from build123d import *

# Parameters (mm, degrees)
SKETCH1_R              = 1.6
BOSS_EXTRUDE1_DEPTH    = 4
CUT_EXTRUDE1_DEPTH     = 44.119746057
R1_CUTOUT_FILLET_R     = 1
R3_OUTER_EDGE_FILLET_R = 3


with BuildPart() as part:
    # Sketch1 → Boss-Extrude1 (new body)
    with BuildSketch(Plane(origin=(0, 0, 0), x_dir=(1, 0, 0), z_dir=(0, 1, 0))):
        Polygon((-40.5, -4.5), (-22.92820323, -4.5), (-16, -0.5), (16, -0.5), (22.92820323, -4.5), (40.5, -4.5), (40.5, 4), (26, 4), (5.5, 14.25), (-5.5, 14.25), (-26, 4), (-40.5, 4), align=None)
        with Locations(Location((-36, 0, 0), (0, 0, 270))):
            Circle(SKETCH1_R, mode=Mode.SUBTRACT)
        with Locations(Location((36, 0, 0), (0, 0, 270))):
            Circle(SKETCH1_R, mode=Mode.SUBTRACT)
        with Locations(Location((0, 10.25, 0), (0, 0, 270))):
            Circle(SKETCH1_R, mode=Mode.SUBTRACT)
    extrude(amount=BOSS_EXTRUDE1_DEPTH)

    # Sketch2 → Cut-Extrude1 (cut, through all)
    with BuildSketch(Plane(origin=(0, 4, 0), x_dir=(1, 0, 0), z_dir=(0, 1, 0))):
        Polygon((-7.655238394, 9.259261842), (-21.173762079, 2.5), (-3.75277675, 2.5), align=None)
        Polygon((-2.742413779, 6.75), (0, 2), (2.742413779, 6.75), align=None)
        Polygon((21.173762079, 2.5), (3.75277675, 2.5), (7.655238394, 9.259261842), align=None)
        Polygon((-31.5, 0), (-21.133974596, 0), (-25.464101615, -2.5), (-31.5, -2.5), align=None)
        Polygon((25.464101615, -2.5), (31.5, -2.5), (31.5, 0), (21.133974596, 0), align=None)
    extrude(amount=-CUT_EXTRUDE1_DEPTH, mode=Mode.SUBTRACT)

    # R1 cutout fillet
    r1_cutout_fillet_edges = [part.edges().sort_by_distance(p)[0] for p in [
        (-25.464101615, 2, 2.5),
        (-31.5, 2, 2.5),
        (-31.5, 2, 0),
        (-21.133974596, 2, 0),
        (25.464101615, 2, 2.5),
        (21.133974596, 2, 0),
        (31.5, 2, 0),
        (31.5, 2, 2.5),
        (7.655238394, 2, -9.259261842),
        (21.173762079, 2, -2.5),
        (3.75277675, 2, -2.5),
        (-2.742413779, 2, -6.75),
        (2.742413779, 2, -6.75),
        (0, 2, -2),
        (-7.655238394, 2, -9.259261842),
        (-3.75277675, 2, -2.5),
        (-21.173762079, 2, -2.5),
    ]]
    fillet(r1_cutout_fillet_edges, radius=R1_CUTOUT_FILLET_R)

    # R3 outer edge fillet
    r3_outer_edge_fillet_edges = [part.edges().sort_by_distance(p)[0] for p in [
        (40.5, 2, -4),
        (40.5, 2, 4.5),
        (22.92820323, 2, 4.5),
        (16, 2, 0.5),
        (-16, 2, 0.5),
        (-22.92820323, 2, 4.5),
        (-40.5, 2, 4.5),
        (-40.5, 2, -4),
        (-26, 2, -4),
        (-5.5, 2, -14.25),
        (5.5, 2, -14.25),
        (26, 2, -4),
    ]]
    fillet(r3_outer_edge_fillet_edges, radius=R3_OUTER_EDGE_FILLET_R)


solid = part.part
Part model, mm, in its own coordinate system. A direction names the side the tool comes from. Give positions to 0.01 mm unless a question says otherwise; leave off trailing zeros. Write each loop counter-clockwise with the first axis right and the second up, starting at its lowest first coordinate (ties: lowest second). Pieces come first, ordered by that corner, then holes.
1) Cut at B-B on z = -10.25. Write the cut outline in (x, y), then the cut area to 3 significant figures.
Resolved:
outline: (-13.5, 0) - (-1.6, 0) - (-1.6, 4) - (-13.5, 4) - close; (1.6, 0) - (13.5, 0) - (13.5, 4) - (1.6, 4) - close
area: 95.2 mm2
2) Pin check, flat tips, straight feed: pin 1 (1.2 mm diameter, centred on x = 33.5, y = 1, fed in from -Z); pin 2 (2 mm diameter, centred on x = -10.5, y = 1.5, fed in from -Z); pin 3 (2 mm diameter, centred on x = 13.5, y = 1, fed in from -Z). Stop position of each tip, or through.
Resolved:
pin 1: stops at z = -4
pin 2: stops at z = -12.25
pin 3: stops at z = -10.75
3) Cut at A-A on x = 0. Write the cut outline in (y, z), then the cut area to 3 significant figures.
Resolved:
outline: (0, -14.25) - (4, -14.25) - (4, -11.85) - (0, -11.85) - close; (0, -8.65) - (4, -8.65) - (4, -6.75) - (0, -6.75) - close; (0, -3) - (4, -3) - (4, 0.5) - (0, 0.5) - close
area: 31.2 mm2
4) Probe L1, parallel to Z at x = 28, y = 2.7; L2, parallel to X at y = 1.85, z = 1; L3, parallel to X at y = 0.85, z = 1.25. List the from-to ranges inside material, lowest first.
Resolved:
L1: z = -4 to 0, 2.5 to 4.5
L2: x = -40.5 to -37.25, -34.75 to -31.5, -23.87 to -16.87, 16.87 to 23.87, 31.5 to 34.75, 37.25 to 40.5
L3: x = -40.5 to -37, -35 to -31.5, -23.9 to -17.3, 17.3 to 23.9, 31.5 to 35, 37 to 40.5
5) Cut at C-C on x = 36. Write the cut outline in (y, z), then the cut area to 3 significant figures.
Resolved:
outline: (0, -4) - (4, -4) - (4, -1.6) - (0, -1.6) - close; (0, 1.6) - (4, 1.6) - (4, 4.5) - (0, 4.5) - close
area: 21.2 mm2
6) Which spindle directions (+Z, -Z, +X, -X, +Y, -Y) get a long thin tool onto all of the face, cutting with end or side? Do faces 4 (the face through (0, 2, 0.5)), 5 (the face through (-26.028, 2.028, -4.078)), 6 (the face through (11, 2, -2.5)). Say none if no direction does.
Resolved:
face 4: +Z, +Y, -Y
face 5: -Z, -X, +Y, -Y
face 6: +Y, -Y
7) Cut at D-D on y = 2.9. State how many separate pieces and enclosed holes the cut face has, then the cut area to 3 significant figures.
Resolved:
separate pieces: 1
enclosed holes: 8
area: 667 mm2
8) Two-plate mould, pull along Z, no slides. Class faces 1 (the face through (32, 2, -4)), 2 (the face through (-22.97, 2.03, 4.4)), 3 (the face through (-5.884, 2.028, -6.191)): released by +Z, released by -Z, zero draft, split by the parting line, or undercut.
Resolved:
face 1: released by -Z
face 2: released by +Z
face 3: undercut
